The listing builds one solid part. Answer for the finished solid, in the listing's coordinates (mm). Give positions to 0.01 mm unless a question says otherwise; leave off trailing zeros. Loops run counter-clockwise (first coordinate to the right, second up) from the corner with the lowest first, then second, coordinate; pieces in that order, holes last. Notation, with made-up numbers: (34, -30) - (39, -30) arc R12 ccw to (39, -24) - close; hole circle Ø9 at (-21, 79). An arc over 180 degrees is marked (long way). Write item = value, one per line. Start each with the question number.
1) Consider probe 1 along Y at (x, z) = (0, -0.25); probe 2 along Y at (x, z) = (-11.5, -4); probe 3 along X at (y, z) = (2.25, 3.25). Determine where each line is inside the solid, lowest interval first.
2) The part is cut by section A-A on x = 0. Write down the section's boundary in (y, z), plus the area to 3 significant figures.
3) The mould has two halves that part along Y. Classify faces 1 (the conical face through (-7.29, -12.77, 6.96)), 2 (the conical face through (-7.42, 12.699, -6.958)), 3 (the cylindrical face through (-1.73, -7.81, 0.11)): +Y half, -Y half, draft (parallel to the pull), parting line (faces both ways), or undercut.
4) The part is cut by section C-C on x = -11.5. Write down the section's boundary in (y, z), plus the area to 3 significant figures.
5) The part is cut by section B-B on z = 4. Write down the section's boundary in (x, y), plus the area to 3 significant figures.
6) Flat-ended cylindrical pins translate along their axes: P1, Ø3, axis at x = 12, z = 0, coming from the -Y side; P2, Ø6, axis at x = -12, z = -3.5, coming from the -Y side; P3, Ø5, axis at y = 7, z = -0.5, coming from the -X side. Find the tip coordinate at first contact, or state that the pin passes through.
from build123d import *

# Parameters (mm, degrees)
HEX_BODY_15_THICK_DEPTH = 7.5
BORE_PROFILE_16_R       = 8
BORE_16_THRU_DEPTH      = 7.5


with BuildPart() as part:
    # Hex Profile 28 AF → Hex Body 15 Thick (new, symmetric)
    with BuildSketch(Plane.XY):
        Polygon((16.165807537, 0), (8.082903769, 14), (-8.082903769, 14), (-16.165807537, 0), (-8.082903769, -14), (8.082903769, -14), align=None)
    extrude(amount=HEX_BODY_15_THICK_DEPTH, both=True)

    # Bore Profile Ø16 → Bore Ø16 Thru (cut, symmetric)
    with BuildSketch(Plane.XY):
        Circle(BORE_PROFILE_16_R)
    extrude(amount=BORE_16_THRU_DEPTH, both=True, mode=Mode.SUBTRACT)

    # Chamfer Profile 2mm → Double-Sided Chamfer 2mm (revolve, cut)
    with BuildSketch(Plane(origin=(0, 0, 0), x_dir=(1, 0, 0), z_dir=(0, 1, 0))):
        Polygon((16.165807537, 7.5), (16.165807537, 5.5), (14.165807537, 7.5), align=None)
        Polygon((16.165807537, -7.5), (16.165807537, -5.5), (14.165807537, -7.5), align=None)
    revolve(axis=Axis((0, 0, 1000), (0, 0, -1)), mode=Mode.SUBTRACT)


solid = part.part
Answer below:
q1.probe_1 = -14 to -8, 8 to 14
q1.probe_2 = -8.08 to 8.08
q1.probe_3 = -14.87 to -7.68, 7.68 to 14.87
q2.outline = (-14, -7.5) - (-8, -7.5) - (-8, 7.5) - (-14, 7.5) - close; (8, -7.5) - (14, -7.5) - (14, 7.5) - (8, 7.5) - close
q2.area = 180 mm2
q3.face_1 = -Y half
q3.face_2 = +Y half
q3.face_3 = undercut
q4.outline = (-8.08, -7.5) - (8.08, -7.5) - (8.08, 7.5) - (-8.08, 7.5) - close
q4.area = 242 mm2
q5.outline = (-16.17, 0) - (-8.08, -14) - (8.08, -14) - (16.17, 0) - (8.08, 14) - (-8.08, 14) - close; hole circle Ø16 at (0, 0)
q5.area = 478 mm2
q6.P1 = -9.81
q6.P2 = -12.41
q6.P3 = -13.57
